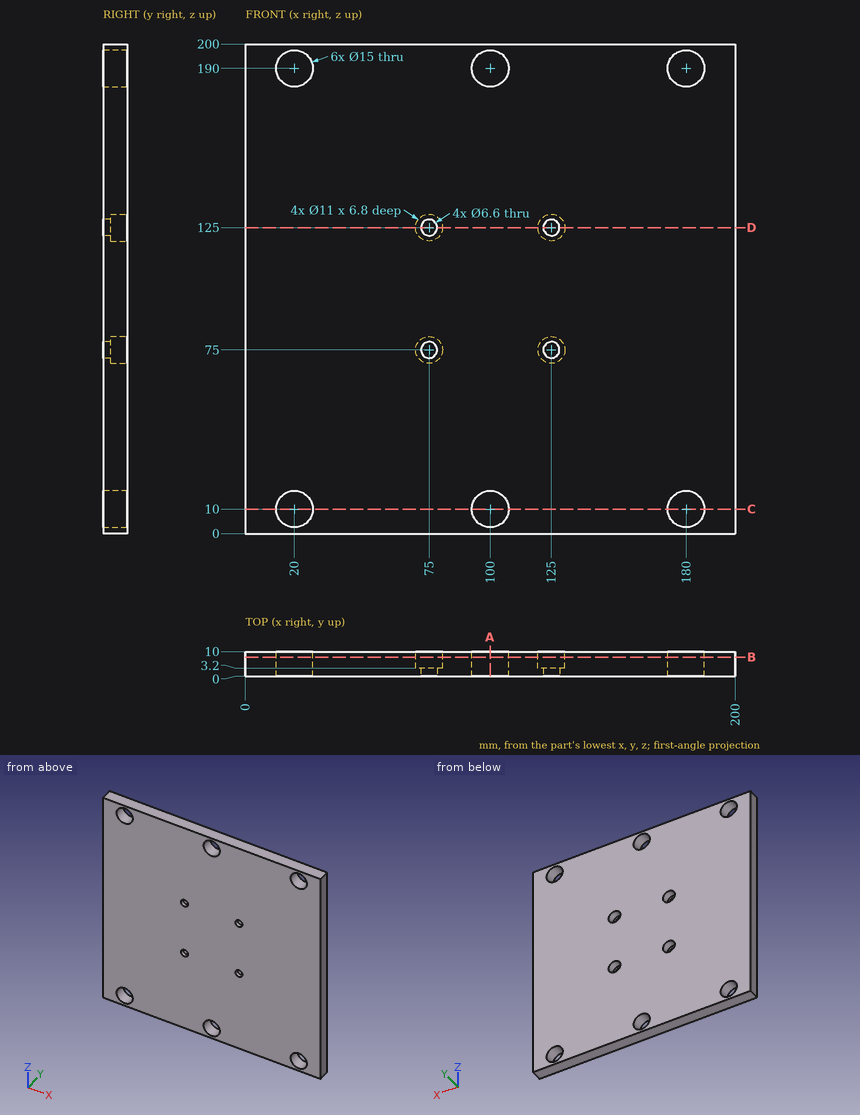
Could you check a few things on this drawing? It's one solid part, dimensions in mm from its lowest x, y, z. Give positions to 0.01 mm unless a question says otherwise; leave off trailing zeros. Order: outer loops, then holes, each group sorted by start corner. A loop starts at its lowest first (then second) coordinate and runs counter-clockwise, first axis right, second up. Notation, with made-up numbers: (41.5, 65.25) - (89.5, 65.25) arc R35 cw to (89.5, 100.25) - close; hole circle Ø1 at (30, -17). An arc over 180 degrees is marked (long way). One line per item, written item: value. Start each with the question number.
1. Imagine slicing it at D-D on z = 125. List the corners of the cut face in (x, y) for me.
2. If I drill on probe 1 along Z at (x, y) = (125, 5.25); probe 2 along Z at (x, y) = (75, 1.7), over which ranges is the centre line in solid material (lowest first)?
3. For P1, Ø12, axis at x = 73, z = 73, coming from the +Y side; P2, Ø7.5, axis at x = 125, z = 75, coming from the +Y side, each with a flat end and sliding along its axis, tell me the tip position at first contact or that it passes through.
4. Imagine slicing it at C-C on z = 10. List the corners of the cut face in (x, y) for me, plus the area to 3 significant figures.
5. Imagine slicing it at A-A on x = 100. List the corners of the cut face in (y, z) for me.
6. Imagine slicing it at B-B on y = 7.75. Give the number of separate pieces and of enclosed holes in the cut face, plus the area to 3 significant figures.
Values:
1. outline: (0, 0) - (71.7, 0) - (71.7, 3.2) - (69.5, 3.2) - (69.5, 10) - (0, 10) - close; (78.3, 0) - (121.7, 0) - (121.7, 3.2) - (119.5, 3.2) - (119.5, 10) - (80.5, 10) - (80.5, 3.2) - (78.3, 3.2) - close; (128.3, 0) - (200, 0) - (200, 10) - (130.5, 10) - (130.5, 3.2) - (128.3, 3.2) - close
2. probe 1: 0 to 69.5, 80.5 to 119.5, 130.5 to 200
2. probe 2: 0 to 71.7, 78.3 to 121.7, 128.3 to 200
3. P1: y = 10
3. P2: y = 3.2
4. outline: (0, 0) - (12.5, 0) - (12.5, 10) - (0, 10) - close; (27.5, 0) - (92.5, 0) - (92.5, 10) - (27.5, 10) - close; (107.5, 0) - (172.5, 0) - (172.5, 10) - (107.5, 10) - close; (187.5, 0) - (200, 0) - (200, 10) - (187.5, 10) - close
4. area: 1,550 mm²
5. outline: (0, 0) - (10, 0) - (10, 2.5) - (0, 2.5) - close; (0, 17.5) - (10, 17.5) - (10, 182.5) - (0, 182.5) - close; (0, 197.5) - (10, 197.5) - (10, 200) - (0, 200) - close
6. separate pieces: 1
6. enclosed holes: 10
6. area: 38,600 mm²
